Work out the finished part from the listing and answer in its coordinate system (mm). Face numbers are marked on the shaded views. A direction names the side the tool comes from. Coordinates: 2 decimals unless noted, no trailing zeros. Write each loop counter-clockwise with the first axis right and the second up, starting at its lowest first coordinate (ties: lowest second). Pieces come first, ordered by that corner, then holes. Notation, with made-up numbers: (11.5, -14.75) - (35.5, -14.75) arc R9 ccw to (35.5, -10.75) - close; hole circle Ø10 at (61.25, 24). An arc over 180 degrees is marked (long way). Use CSV: the item, a comma, the result in double quotes. Start each with the question number.
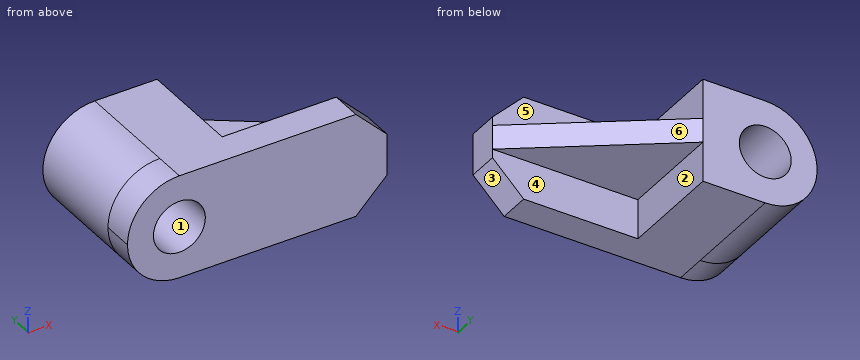
from build123d import *

# Parameters (mm, degrees)
BASE_PLATE_DEPTH      = 9
BASE_END_CUT_DEPTH    = 9
UPRIGHT_START         = 30
UPRIGHT_BOSS_SKETCH_R = 7.5
UPRIGHT_BOSS_DEPTH    = 30
SUPPORT_RIB_DEPTH     = 3.5
BOSS_BORE_SKETCH_R    = 7.5
BOSS_BORE_DEPTH       = 57.144901817


with BuildPart() as part:
    # Base Plate Sketch → Base Plate (new body)
    with BuildSketch(Plane(origin=(0, 0, 0), x_dir=(1, 0, 0), z_dir=(0, 1, 0))):
        Polygon((28.5, 15), (37.5, 6), (37.5, -6), (28.5, -15), (-37.5, -15), (-37.5, 15), align=None)
    extrude(amount=BASE_PLATE_DEPTH)

    # Base End Cut Sketch → Base End Cut (cut)
    with BuildSketch(Plane(origin=(0, 9, 0), x_dir=(1, 0, 0), z_dir=(0, 1, 0))):
        with BuildLine():
            Line((-37.5, 1.12e-07), (-37.5, -15))
            Line((-37.5, -15), (-22.5, -15))
            ThreePointArc((-22.5, -15), (-33.106601757, -10.606601678), (-37.5, 1.12e-07))
        make_face()
        with BuildLine():
            Line((-37.5, 15), (-37.5, 1.12e-07))
            ThreePointArc((-37.5, 1.12e-07), (-33.106601678, 10.606601757), (-22.5, 15))
            Line((-22.5, 15), (-37.5, 15))
        make_face()
    extrude(amount=-BASE_END_CUT_DEPTH, mode=Mode.SUBTRACT)

    # Upright Boss Sketch → Upright Boss (add)
    with BuildSketch(Plane(origin=(0, 9, 0), x_dir=(1, 0, 0), z_dir=(0, 1, 0)).offset(UPRIGHT_START)):
        with BuildLine():
            Line((-4.5, 15), (-22.5, 15))
            ThreePointArc((-22.5, 15), (-37.5, 0), (-22.5, -15))
            Line((-22.5, -15), (-4.5, -15))
            Line((-4.5, -15), (-4.5, 15))
        make_face()
        with Locations(Location((-22.5, 0, 0), (0, 0, 270))):
            Circle(UPRIGHT_BOSS_SKETCH_R, mode=Mode.SUBTRACT)
    extrude(amount=-UPRIGHT_BOSS_DEPTH)

    # Support Rib Sketch → Support Rib (add, symmetric)
    with BuildSketch(Plane.XY):
        Polygon((-4.5, 39), (37.5, 9), (-4.5, 9), align=None)
    extrude(amount=SUPPORT_RIB_DEPTH, both=True)

    # Boss Bore Sketch → Boss Bore (cut, through all)
    with BuildSketch(Plane(origin=(0, 39, 0), x_dir=(1, 0, 0), z_dir=(0, 1, 0))):
        with Locations(Location((-22.5, 0, 0), (0, 0, 270))):
            Circle(BOSS_BORE_SKETCH_R)
    extrude(amount=-BOSS_BORE_DEPTH, mode=Mode.SUBTRACT)


solid = part.part
Item 1: A cutting plane is placed at B-B (z = 1). Determine the outline of the cut face in (x, y), then the cut area to 3 significant figures.
Item 2: A cutting plane is placed at A-A (y = 3.5). Determine the outline of the cut face in (x, z).
Item 3: A cutting plane is placed at C-C (x = -26). Determine the outline of the cut face in (y, z), then the cut area to 3 significant figures.
Item 4: Straight lines are drawn through the part: probe 1 along Z at (x, y) = (-18, 2.5); probe 2 along Z at (x, y) = (13, 19); probe 3 along X at (y, z) = (33, -4). For each, find the intervals that lie inside material, in ascending order. Write a range as [from, to].
Item 5: A cutting plane is placed at D-D (x = 30.5). Determine the outline of the cut face in (y, z).
Item 6: Determine the mould class of the marked faces 1, 2 and 3 for opening direction Z: +Z half, -Z half, draft (parallel to the pull), parting line (faces both ways), or undercut.
Item 7: Each of these flat-tipped pins is pushed along its axis until it touches: pin 1 (5 mm diameter, centred on x = -0.5, z = -4, fed in from +Y); pin 2 (6 mm diameter, centred on x = 20.5, z = 10.5, fed in from +Y); pin 3 (10 mm diameter, centred on x = 27, z = -1.5, fed in from +Y). Where does it stop, or does it pass through?
Item 8: Which of the six approach directions +Z, -Z, +X, -X, +Y, -Y give full straight-line access (tool end or side, diameter ignored) to the marked faces 4, 5 and 6?
Calculated:
1,outline,"(-37.47, 0) - (-29.93, 0) - (-29.93, 39) - (-37.47, 39) - close; (-15.07, 0) - (37.5, 0) - (37.5, 9) - (-4.5, 39) - (-15.07, 39) - close"
1,area,"1,710 mm²"
2,outline,"(-22.5, -15) - (28.5, -15) - (37.5, -6) - (37.5, 6) - (28.5, 15) - (-22.5, 15) arc R15 ccw to start; hole circle Ø15 at (-22.5, 0)"
3,outline,"(0, -14.59) - (39, -14.59) - (39, -6.63) - (0, -6.63) - close; (0, 6.63) - (39, 6.63) - (39, 14.59) - (0, 14.59) - close"
3,area,"620 mm²"
4,probe 1,"z = [-15, -6], [6, 15]"
4,probe 2,"z = [-3.5, 3.5]"
4,probe 3,"x = [-36.96, -28.84], [-16.16, -4.5]"
5,outline,"(0, -13) - (9, -13) - (9, -3.5) - (14, -3.5) - (14, 3.5) - (9, 3.5) - (9, 13) - (0, 13) - close"
6,face 1,"undercut"
6,face 2,"draft"
6,face 3,"-Z half"
7,pin 1,"stops at y = 37.89"
7,pin 2,"stops at y = 9"
7,pin 3,"stops at y = 20.07"
8,face 4,"-Z, +X, +Y"
8,face 5,"+Z, +X, +Y"
8,face 6,"+Z, -Z, +X, +Y"
